```python
from build123d import *

# Parameters (mm, degrees)
SKETCH2_W               = 13.5
SKETCH2_H               = 13.5
CUT_EXTRUDE1_DEPTH      = 9
CHAMFER1_SIZE           = 1
CUT_EXTRUDE2_DEPTH      = 35.073450075
CUT_EXTRUDE2_DEPTH_BACK = 35.073450075
CHAMFER2_SIZE           = 0.5


with BuildPart() as part:
    # Sketch1 → Revolve1 (revolve)
    with BuildSketch(Plane(origin=(0, 0, 0), x_dir=(1, 0, 0), z_dir=(0, 1, 0))):
        Polygon((0, -3), (14, -3), (14, 0), (-19, 0), (-19, -20), (0, -20), align=None)
    revolve(axis=Axis((-19, 0, 0), (1, 0, 0)))

    # Sketch2 → Cut-Extrude1 (cut)
    with BuildSketch(Plane(origin=(-19, 0, 0), x_dir=(0, 0, -1), z_dir=(1, 0, 0))):
        Rectangle(SKETCH2_W, SKETCH2_H)
    extrude(amount=CUT_EXTRUDE1_DEPTH, mode=Mode.SUBTRACT)

    # Chamfer1
    chamfer1_edges = [part.edges().sort_by_distance(p)[0] for p in [
        (-19, 0, 6.75),
        (-19, -6.75, 0),
        (-19, 0, -6.75),
        (-19, 6.75, 0),
    ]]
    chamfer(chamfer1_edges, length=CHAMFER1_SIZE)

    # Sketch3 → Cut-Extrude2 (cut, two sides: drawn at the far end of the back side and taken through both)
    with BuildSketch(Plane(origin=(0, 0, 0), x_dir=(1, 0, 0), z_dir=(0, 1, 0)).offset(-CUT_EXTRUDE2_DEPTH_BACK)):
        with BuildLine():
            Line((2, 1), (4, 1))
            ThreePointArc((4, 1), (5, 0), (4, -1))
            Line((4, -1), (2, -1))
            ThreePointArc((2, -1), (1, 0), (2, 1))
        make_face()
    extrude(amount=CUT_EXTRUDE2_DEPTH + CUT_EXTRUDE2_DEPTH_BACK, mode=Mode.SUBTRACT)

    # Chamfer2
    chamfer2_edges = [part.edges().sort_by_distance(p)[0] for p in [
        (14, 0, -3),
    ]]
    chamfer(chamfer2_edges, length=CHAMFER2_SIZE)


solid = part.part
```
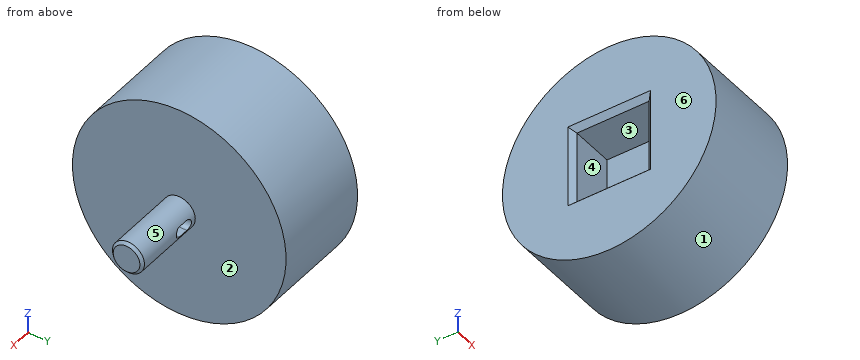
Model file for the job. Use its own axes, mm. Face numbers are marked on the shaded views. A direction names the side the tool comes from. Give positions to 0.01 mm unless a question says otherwise; leave off trailing zeros. Loops run counter-clockwise (first coordinate to the right, second up) from the corner with the lowest first, then second, coordinate; pieces in that order, holes last. Notation, with made-up numbers: M 17.25,-15.5 L 68.25,-15.5 A24 ccw 68.25,-0.5 Z; hole C 37.25,41.25 d11. An arc over 180 degrees is marked long. Use one line per item in the form item = value.
Item 1: Slice it at B-B on z = -12. List the corners of the cut face in (x, y).
Filled in:
outline = M -19,-16 L 0,-16 L 0,16 L -19,16 Z
Item 2: Flat gauge pins, fed straight in: pin 1 Ø2 at (x, y) = (-1, 3) entering from +Z; pin 2 Ø2.5 at (x, z) = (-16, 0.5) entering from -Y; pin 3 Ø12 at (x, y) = (-6.5, 9) entering from +Z; pin 4 Ø3 at (x, z) = (2.5, 9) entering from -Y. Where does each tip first touch, or does it go through?
Filled in:
pin_1 = 19.9
pin_2 = -20
pin_3 = 19.77
pin_4 = through
Item 3: Two-plate mould, pull along Y, no slides. Class the marked faces 1, 2 and 3: released by +Y, released by -Y, zero draft, split by the parting line, or undercut.
Filled in:
face_1 = split by the parting line
face_2 = zero draft
face_3 = undercut
Item 4: Which spindle directions (+Z, -Z, +X, -X, +Y, -Y) get a long thin tool onto all of the face, cutting with end or side? Do the marked faces 4, 5 and 6. Say none if no direction does.
Filled in:
face_4 = -X
face_5 = +X
face_6 = +Z, -Z, -X, +Y, -Y
Item 5: Drill centre lines: L1, parallel to X at y = 10.5, z = -8; L2, parallel to Z at x = -14.5, y = 4.5; L3, parallel to Z at x = -12.5, y = 10.5. Where is each one in solid material? Low to high.
Filled in:
L1 = -19 to 0
L2 = -19.49 to -6.75, 6.75 to 19.49
L3 = -17.02 to 17.02
Item 6: Slice it at C-C on y = 6. List the corners of the cut face in (x, z).
Filled in:
outline = M -19,-19.08 L 0,-19.08 L 0,19.08 L -19,19.08 L -19,7.75 L -18,6.75 L -10,6.75 L -10,-6.75 L -18,-6.75 L -19,-7.75 Z
Item 7: Slice it at D-D on x = 7.5. List the corners of the cut face in (y, z).
Filled in:
outline = C 0,0 d6
Item 8: Slice it at A-A on x = -14.5. List the corners of the cut face in (y, z), and give its area (3 significant figures).
Filled in:
outline = C 0,0 d40; hole M -6.75,-6.75 L 6.75,-6.75 L 6.75,6.75 L -6.75,6.75 Z
area = 1,070 mm^2
